The model under review builds one solid part; all positions refer to its coordinate system, in mm. Coordinates: 2 decimals unless noted, no trailing zeros. Write each loop counter-clockwise with the first axis right and the second up, starting at its lowest first coordinate (ties: lowest second). Pieces come first, ordered by that corner, then holes. Notation, with made-up numbers: (53, 51.25) -> (67, 51.25) arc R29 cw to (67, 86.25) -> close; hole circle Ø3 at (57.25, 0). An arc over 180 degrees is marked (long way). Write each question's results on one line, items separated by ' | '.
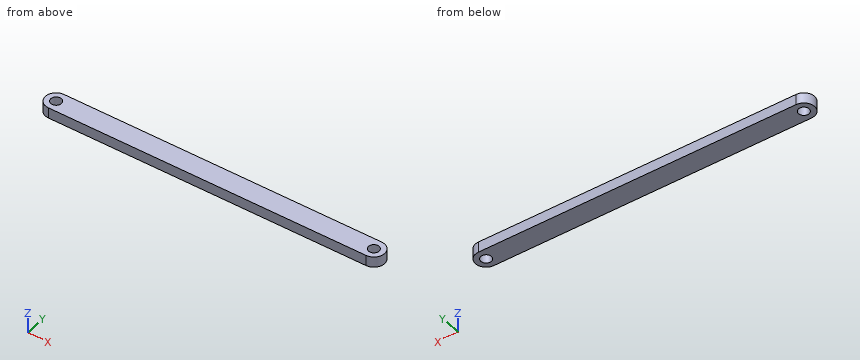
```python
from build123d import *

# Parameters (mm, degrees)
SKETCH1_R           = 5
BOSS_EXTRUDE1_DEPTH = 10


with BuildPart() as part:
    # Sketch1 → Boss-Extrude1 (new body)
    with BuildSketch(Plane.XY):
        with BuildLine():
            Line((-0.109854152, 9.999396585), (299.8720434, 13.295021139))
            ThreePointArc((299.8720434, 13.295021139), (309.981294137, 3.405478706), (300.091751704, -6.703772031))
            Line((300.091751704, -6.703772031), (0.109854152, -9.999396585))
            ThreePointArc((0.109854152, -9.999396585), (-9.999396585, -0.109854152), (-0.109854152, 9.999396585))
        make_face()
        with Locations((299.981897552, 3.295624554)):
            Circle(SKETCH1_R, mode=Mode.SUBTRACT)
        Circle(SKETCH1_R, mode=Mode.SUBTRACT)
    extrude(amount=BOSS_EXTRUDE1_DEPTH)


solid = part.part
```
Q1. Add section B-B (x = 87.5). Write out the cut boundary in (y, z).
Solution:
outline: (-9.04, 0) -> (10.96, 0) -> (10.96, 10) -> (-9.04, 10) -> close
Q2. Add section A-A (z = 6.5). Write out the cut boundary in (x, y), plus the area to 3 significant figures.
Solution:
outline: (-0.11, 10) arc R10 ccw to (0.11, -10) -> (300.09, -6.7) arc R10 ccw to (299.87, 13.3) -> close; hole circle Ø10 at (0, 0); hole circle Ø10 at (299.98, 3.3) | area: 6,160 mm²
Q3. For line 1 (X direction, y = 0.75, z = 8.75); line 2 (X direction, y = -1, z = 7.75); line 3 (Y direction, x = 274, z = 2.25), list the stretches that pass through material, from the lowest coordinate up. Write a range as from..to.
Solution:
line 1: -9.97..-4.94, 4.94..295.68, 304.29..309.65 | line 2: -9.95..-4.9, 4.9..297.42, 302.54..309.01 | line 3: -6.99..13.01
Q4. Clearance check with flat-ended pins moving along their axes: P1, Ø3, axis at x = 220.5, z = 7, coming from the -Y side; P2, Ø3, axis at y = 10, z = 2.5, coming from the -X side; P3, Ø2, axis at y = -6, z = 2, coming from the +X side. State where each tip first meets the part, or that it passes through.
Solution:
P1: y = -7.59 | P2: x = -5.27 | P3: x = 305.57
